Check sheet for the drawn part. Datum: minimum x, y, z corner. Units: mm. Give positions to 0.01 mm unless a question says otherwise; leave off trailing zeros. Write each loop counter-clockwise with the first axis right and the second up, starting at its lowest first coordinate (ties: lowest second). Pieces come first, ordered by that corner, then holes.
(1) Cross-section at A-A (x = 90). Record the boundary of the cut face in (y, z), and give its area (3 significant figures).
(2) Depth check by flat-ended pin: P1, Ø4, axis at y = 66.5, z = 118.5, coming from the -X side. Enter the tip coordinate at first touch or a pass-through.
(3) Mould release check, pull along Z, two halves, no side actions. Record for the marked faces 1, 2, 3 and 4: +Z half, -Z half, draft (parallel to the pull), parting line (faces both ways), or undercut.
(4) Cross-section at C-C (y = 20). Record the boundary of the cut face in (x, z).
(5) Thickness scan on line 1 along X through (y, z) = (67.5, 75); line 2 along Z through (x, y) = (210, 70); line 3 along X through (y, z) = (55, 87.5). Record the ranges inside material, lowest first.
(6) Cross-section at B-B (z = 75). Record the boundary of the cut face in (x, y), and give its area (3 significant figures).
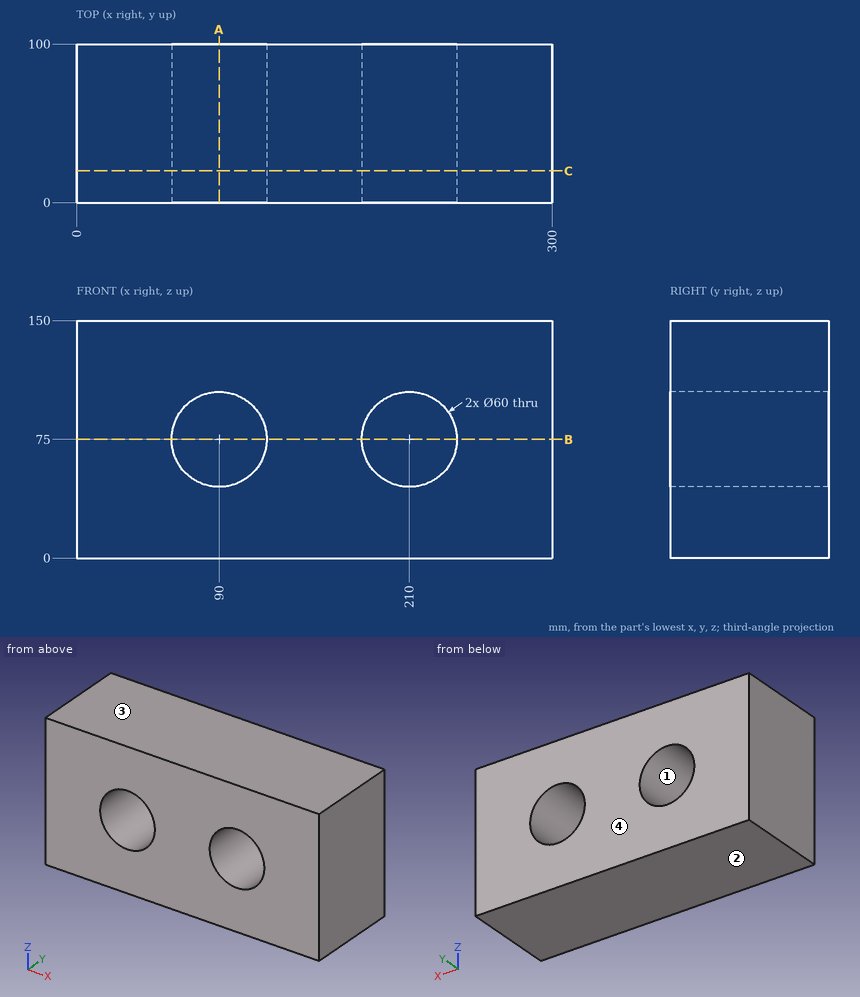
Reply:
1. outline: (0, 0) - (100, 0) - (100, 45) - (0, 45) - close; (0, 105) - (100, 105) - (100, 150) - (0, 150) - close
1. area: 9,000 mm2
2. P1: stops at x = 0
3. face 1: undercut
3. face 2: -Z half
3. face 3: +Z half
3. face 4: draft
4. outline: (0, 0) - (300, 0) - (300, 150) - (0, 150) - close; hole circle Ø60 at (90, 75); hole circle Ø60 at (210, 75)
5. line 1: x = 0 to 60, 120 to 180, 240 to 300
5. line 2: z = 0 to 45, 105 to 150
5. line 3: x = 0 to 62.73, 117.27 to 182.73, 237.27 to 300
6. outline: (0, 0) - (60, 0) - (60, 100) - (0, 100) - close; (120, 0) - (180, 0) - (180, 100) - (120, 100) - close; (240, 0) - (300, 0) - (300, 100) - (240, 100) - close
6. area: 18,000 mm2
